Read the model definition and answer for the solid it produces. Units are mm, in the model's axes. Face numbers are marked on the shaded views. A direction names the side the tool comes from. Round coordinates to 2 decimals unless told otherwise and drop trailing zeros. Write each loop counter-clockwise with the first axis right and the second up, starting at its lowest first coordinate (ties: lowest second). Pieces come first, ordered by that corner, then holes.
from build123d import *

# Parameters (mm, degrees)
SKETCH_1_W          = 250
SKETCH_1_H          = 55
EXTRUDE_1_DEPTH     = 150
SKETCH_2_W          = 230
SKETCH_2_H          = 130
CUT_EXTRUDE_1_DEPTH = 45
SKETCH_4_W          = 65
SKETCH_4_H          = 45
CUT_EXTRUDE_2_DEPTH = 223.093390385
SKETCH_10_R         = 2.1
CUT_EXTRUDE_8_DEPTH = 17.7


with BuildPart() as part:
    # 草图1 → 凸台-拉伸1 (new body)
    with BuildSketch(Plane.XY):
        with Locations((-32.481662592, 40.947432763)):
            Rectangle(SKETCH_1_W, SKETCH_1_H)
    extrude(amount=EXTRUDE_1_DEPTH)

    # 草图2 → 切除-拉伸1 (cut)
    with BuildSketch(Plane.XZ.offset(-13.447432763)):
        with Locations((-32.481662592, 75)):
            Rectangle(SKETCH_2_W, SKETCH_2_H)
    extrude(amount=-CUT_EXTRUDE_1_DEPTH, mode=Mode.SUBTRACT)

    # 草图4 → 切除-拉伸2 (cut, through all)
    with BuildSketch(Plane.XZ.offset(-58.447432763)):
        with Locations((10.018337408, 47.5)):
            Rectangle(SKETCH_4_W, SKETCH_4_H)
    extrude(amount=-CUT_EXTRUDE_2_DEPTH, mode=Mode.SUBTRACT)

    # 草图10 → 切除-拉伸8 (cut)
    with BuildSketch(Plane(origin=(971.262341276, 76.147432763, 1019.143932915), x_dir=(1, 0, 0), z_dir=(0, 1, 0))):
        with Locations(Location((-1055.250263055, 981.942263912, 0), (0, 0, 270))):
            Circle(SKETCH_10_R)
        with Locations(Location((-1055.250263055, 958.292263912, 0), (0, 0, 270))):
            Circle(SKETCH_10_R)
        with Locations(Location((-1014.250263055, 958.292263912, 0), (0, 0, 270))):
            Circle(SKETCH_10_R)
        with Locations(Location((-1014.250263055, 981.942263912, 0), (0, 0, 270))):
            Circle(SKETCH_10_R)
    extrude(amount=-CUT_EXTRUDE_8_DEPTH, mode=Mode.SUBTRACT)


solid = part.part
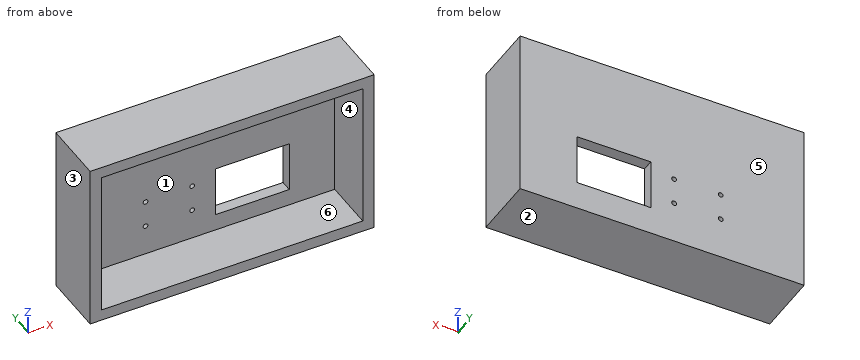
Q1. Section C-C (y = 53) is taken. Determine the outline of the cut face in (x, z), then the cut area to 3 significant figures.
Verdict:
outline: (-157.48, 0) - (92.52, 0) - (92.52, 150) - (-157.48, 150) - close; hole (-147.48, 10) - (82.52, 10) - (82.52, 140) - (-147.48, 140) - close
area: 7,600 mm2
Q2. Section B-B (x = 50) is taken. Determine the outline of the cut face in (y, z).
Verdict:
outline: (13.45, 0) - (68.45, 0) - (68.45, 150) - (13.45, 150) - (13.45, 140) - (58.45, 140) - (58.45, 10) - (13.45, 10) - close
Q3. A flat-ended cylindrical pin translates along its axis: pin 1 Ø10 at (x, z) = (-97.5, 112.5) entering from -Y. Find the tip coordinate at first contact, or state that the pin passes through.
Verdict:
pin 1: stops at y = 58.45
Q4. Section A-A (z = 42.5) is taken. Determine the outline of the cut face in (x, y), then the cut area to 3 significant figures.
Verdict:
outline: (-157.48, 13.45) - (-147.48, 13.45) - (-147.48, 58.45) - (-22.48, 58.45) - (-22.48, 68.45) - (-157.48, 68.45) - close; (42.52, 58.45) - (82.52, 58.45) - (82.52, 13.45) - (92.52, 13.45) - (92.52, 68.45) - (42.52, 68.45) - close
area: 2,750 mm2
Q5. Which of the six approach directions +Z, -Z, +X, -X, +Y, -Y give full straight-line access (tool end or side, diameter ignored) to the marked faces 5 and 6?
Verdict:
face 5: +Z, -Z, +X, -X, +Y
face 6: -Y
Q6. Section D-D (z = 16) is taken. Determine the outline of the cut face in (x, y).
Verdict:
outline: (-157.48, 13.45) - (-147.48, 13.45) - (-147.48, 58.45) - (82.52, 58.45) - (82.52, 13.45) - (92.52, 13.45) - (92.52, 68.45) - (-157.48, 68.45) - close
Q7. Determine the mould class of the marked faces 1, 2, 3 and 4 for opening direction X: pulls with the +X half, pulls with the -X half, needs draft (parallel to the pull), parting line crosses it, or undercut.
Verdict:
face 1: undercut
face 2: needs draft
face 3: pulls with the -X half
face 4: undercut
Q8. Straight lines are drawn through the part: probe 1 along X at (y, z) = (50.5, 113); probe 2 along Z at (x, y) = (61, 41); probe 3 along X at (y, z) = (63.5, 42). For each, find the intervals that lie inside material, in ascending order.
Verdict:
probe 1: x = -157.48 to -147.48, 82.52 to 92.52
probe 2: z = 0 to 10, 140 to 150
probe 3: x = -157.48 to -22.48, 42.52 to 92.52
